```python
from build123d import *

# Parameters (mm, degrees)
BOSS_EXTRUDE1_DEPTH      = 4.7625
BOSS_EXTRUDE1_DEPTH_BACK = 4.7625
SKETCH1_R                = 3.9624
BOSS_EXTRUDE2_DEPTH      = 14.2875
BOSS_EXTRUDE2_DEPTH_BACK = 14.2875
BOSS_EXTRUDE2_START      = -4.7625
SKETCH2_R                = 3.175


with BuildPart() as part:
    # Sketch1 → Boss-Extrude1 (new, two sides: drawn at the far end of the back side and taken through both)
    with BuildSketch(Plane.XY.offset(-BOSS_EXTRUDE1_DEPTH_BACK)):
        Circle(SKETCH1_R)
    extrude(amount=BOSS_EXTRUDE1_DEPTH + BOSS_EXTRUDE1_DEPTH_BACK)

    # Sketch2 → Boss-Extrude2 (add, two sides: drawn at the far end of the back side and taken through both)
    with BuildSketch(Plane.XY.offset(4.7625).offset(BOSS_EXTRUDE2_START - BOSS_EXTRUDE2_DEPTH_BACK)):
        Circle(SKETCH2_R)
    extrude(amount=BOSS_EXTRUDE2_DEPTH + BOSS_EXTRUDE2_DEPTH_BACK)


solid = part.part
```
Could you check a few things on this model? Use its own coordinates, in mm. A direction names the side the tool comes from. Coordinates: 2 decimals unless noted, no trailing zeros. Loops run counter-clockwise (first coordinate to the right, second up) from the corner with the lowest first, then second, coordinate; pieces in that order, holes last.
1) Please list where these lines run through material, in increasing order: line 1 along Z through (x, y) = (1.5, -3.5); line 2 along X through (y, z) = (0, -7) (3 decimals); line 3 along Y through (x, z) = (2.75, -2.25).
Reported:
line 1: z = -4.76 to 4.76
line 2: x = -3.175 to 3.175
line 3: y = -2.85 to 2.85
2) Imagine slicing it at A-A (y = 0). List the corners of the cut face in (x, z) for me (1 decimal).
Reported:
outline: (-4, -4.8) - (-3.2, -4.8) - (-3.2, -14.3) - (3.2, -14.3) - (3.2, -4.8) - (4, -4.8) - (4, 4.8) - (3.2, 4.8) - (3.2, 14.3) - (-3.2, 14.3) - (-3.2, 4.8) - (-4, 4.8) - close
3) Imagine slicing it at C-C (z = 3.5). List the corners of the cut face in (x, y) for me.
Reported:
outline: circle Ø7.92 at (0, 0)
4) Will these pins go through, and if not, where does the flat tip stop? pin 1 Ø4 at (y, z) = (-3, 5) entering from +X; pin 2 Ø1.5 at (x, z) = (-2.5, 2.5) entering from +Y (3 decimals); pin 3 Ø1.5 at (x, z) = (2, 0) entering from -Y.
Reported:
pin 1: stops at x = 3.83
pin 2: stops at y = 3.555
pin 3: stops at y = -3.76
5) Imagine slicing it at D-D (z = 7.5). List the corners of the cut face in (x, y) for me (3 decimals), and give its area (3 significant figures).
Reported:
outline: circle Ø6.35 at (0, 0)
area: 31.7 mm2
6) Which directions (+Z, -Z, +X, -X, +Y, -Y) give clear straight access to the entire face, cutting with the end or side of a thin tool? Please do faces 1 (the face through (-0.69, -3.1, 9.46)), 2 (the face through (-3, -2, -4.762)), 3 (the face through (-0.52, 3.93, -0.07)).
Reported:
face 1: +Z
face 2: -Z
face 3: +Z, -Z
